```python
from build123d import *

# Parameters (mm, degrees)
SKETCH1_W           = 18
SKETCH1_H           = 56
BOSS_EXTRUDE1_DEPTH = 10
SKETCH2_W           = 6
SKETCH2_H           = 56
CUT_EXTRUDE1_DEPTH  = 1.5
HOLE1_D             = 3.242
HOLE1_DEPTH         = 6
HOLE1_CSINK_D       = 4
HOLE1_CSINK_ANGLE   = 90
HOLE1_TIP           = 0.935884786
HOLE2_D             = 3.242
HOLE2_DEPTH         = 6
HOLE2_CSINK_D       = 4
HOLE2_CSINK_ANGLE   = 90
HOLE2_TIP           = 0.935884786
HOLE3_D             = 3.242
HOLE3_DEPTH         = 6
HOLE3_CSINK_D       = 4
HOLE3_CSINK_ANGLE   = 90
HOLE3_TIP           = 0.935884786
HOLE4_D             = 3.242
HOLE4_DEPTH         = 6
HOLE4_CSINK_D       = 4
HOLE4_CSINK_ANGLE   = 90
HOLE4_TIP           = 0.935884786
SKETCH15_R          = 5
SKETCH15_R_2        = 4.5
CUT_EXTRUDE2_DEPTH  = 1
CUT_EXTRUDE3_DEPTH  = 4.33
SKETCH17_R          = 3
SKETCH17_R_2        = 2.5
CUT_EXTRUDE4_DEPTH  = 1
CUT_EXTRUDE5_DEPTH  = 3


with BuildPart() as part:
    # Sketch1 → Boss-Extrude1 (new body)
    with BuildSketch(Plane.XY.offset(9)):
        Rectangle(SKETCH1_W, SKETCH1_H)
    extrude(amount=BOSS_EXTRUDE1_DEPTH)

    # Sketch2 → Cut-Extrude1 (cut)
    with BuildSketch(Plane.XY.offset(9)):
        Rectangle(SKETCH2_W, SKETCH2_H)
    extrude(amount=CUT_EXTRUDE1_DEPTH, mode=Mode.SUBTRACT)

    # Sketch3 → Revolve1 (revolve)
    with BuildSketch(Plane(origin=(0, 0, 0), x_dir=(0, 0, -1), z_dir=(1, 0, 0)), mode=Mode.PRIVATE) as revolve1_sk:
        Polygon((-14, 12.5), (-14, 16.5), (40, 16.5), (40, 20), (45, 20), (45, 12.5), align=None)
    revolve(revolve1_sk.sketch.rotate(Axis((0, 12.5, -45), (0, 0, 1)), 270), axis=Axis((0, 12.5, -45), (0, 0, 1)))

    # Sketch4 → Revolve2 (revolve)
    with BuildSketch(Plane(origin=(0, 0, 0), x_dir=(0, 0, -1), z_dir=(1, 0, 0)), mode=Mode.PRIVATE) as revolve2_sk:
        Polygon((-14, -12.5), (-14, -8.5), (40, -8.5), (40, -5), (45, -5), (45, -12.5), align=None)
    revolve(revolve2_sk.sketch.rotate(Axis((0, -12.5, -45), (0, 0, 1)), 270), axis=Axis((0, -12.5, -45), (0, 0, 1)))

    # Sketch5 → Cut-Revolve1 (revolve, cut)
    with BuildSketch(Plane(origin=(0, 0, 0), x_dir=(0, 0, -1), z_dir=(1, 0, 0)), mode=Mode.PRIVATE) as cut_revolve1_sk:
        Polygon((-19, 22.5), (-19, 25), (-18.567, 24.567), (-10.933, 24.567), (-10.5, 25), (-10.5, 22.5), align=None)
    revolve(cut_revolve1_sk.sketch.rotate(Axis((0, 22.5, 10.5), (0, 0, 1)), 270), axis=Axis((0, 22.5, 10.5), (0, 0, 1)), mode=Mode.SUBTRACT)

    # Sketch6 → Cut-Revolve2 (revolve, cut)
    with BuildSketch(Plane(origin=(0, 0, 0), x_dir=(0, 0, -1), z_dir=(1, 0, 0)), mode=Mode.PRIVATE) as cut_revolve2_sk:
        Polygon((-19, -22.5), (-19, -20), (-18.567, -20.433), (-10.933, -20.433), (-10.5, -20), (-10.5, -22.5), align=None)
    revolve(cut_revolve2_sk.sketch.rotate(Axis((0, -22.5, 10.5), (0, 0, 1)), 270), axis=Axis((0, -22.5, 10.5), (0, 0, 1)), mode=Mode.SUBTRACT)

    # Hole1
    with Locations(Plane.ZY.offset(9)):
        with Locations((14, 22.5)):
            CounterSinkHole(HOLE1_D / 2, HOLE1_CSINK_D / 2, depth=HOLE1_DEPTH, counter_sink_angle=HOLE1_CSINK_ANGLE)
            with Locations((0, 0, -(HOLE1_DEPTH + HOLE1_TIP / 2))):  # 120° drill point
                Cone(0, HOLE1_D / 2, HOLE1_TIP, mode=Mode.SUBTRACT)

    # Hole2
    with Locations(Plane.ZY.offset(9)):
        with Locations((14, -22.5)):
            CounterSinkHole(HOLE2_D / 2, HOLE2_CSINK_D / 2, depth=HOLE2_DEPTH, counter_sink_angle=HOLE2_CSINK_ANGLE)
            with Locations((0, 0, -(HOLE2_DEPTH + HOLE2_TIP / 2))):  # 120° drill point
                Cone(0, HOLE2_D / 2, HOLE2_TIP, mode=Mode.SUBTRACT)

    # Hole3
    with Locations(Plane(origin=(9, 0, 0), x_dir=(0, 0, -1), z_dir=(1, 0, 0))):
        with Locations((-14, 22.5)):
            CounterSinkHole(HOLE3_D / 2, HOLE3_CSINK_D / 2, depth=HOLE3_DEPTH, counter_sink_angle=HOLE3_CSINK_ANGLE)
            with Locations((0, 0, -(HOLE3_DEPTH + HOLE3_TIP / 2))):  # 120° drill point
                Cone(0, HOLE3_D / 2, HOLE3_TIP, mode=Mode.SUBTRACT)

    # Hole4
    with Locations(Plane(origin=(9, 0, 0), x_dir=(0, 0, -1), z_dir=(1, 0, 0))):
        with Locations((-14, -22.5)):
            CounterSinkHole(HOLE4_D / 2, HOLE4_CSINK_D / 2, depth=HOLE4_DEPTH, counter_sink_angle=HOLE4_CSINK_ANGLE)
            with Locations((0, 0, -(HOLE4_DEPTH + HOLE4_TIP / 2))):  # 120° drill point
                Cone(0, HOLE4_D / 2, HOLE4_TIP, mode=Mode.SUBTRACT)

    # Sketch15 → Cut-Extrude2 (cut)
    with BuildSketch(Plane.XY.offset(19)):
        with Locations((0, -12.5)):
            Circle(SKETCH15_R)
        with Locations((0, -12.5)):
            Circle(SKETCH15_R_2, mode=Mode.SUBTRACT)
    extrude(amount=-CUT_EXTRUDE2_DEPTH, mode=Mode.SUBTRACT)

    # Sketch16 → Cut-Extrude3 (cut)
    with BuildSketch(Plane.XY.offset(19)):
        Polygon((-2.499926666, -12.5), (-1.249963333, -14.665), (1.249963333, -14.665), (2.499926666, -12.5), (1.249963333, -10.335), (-1.249963333, -10.335), align=None)
    extrude(amount=-CUT_EXTRUDE3_DEPTH, mode=Mode.SUBTRACT)

    # Sketch17 → Cut-Extrude4 (cut)
    with BuildSketch(Plane(origin=(9, 0, 0), x_dir=(0, 0, -1), z_dir=(1, 0, 0))):
        with Locations((-14, 12.5)):
            Circle(SKETCH17_R)
        with Locations((-14, 12.5)):
            Circle(SKETCH17_R_2, mode=Mode.SUBTRACT)
    extrude(amount=-CUT_EXTRUDE4_DEPTH, mode=Mode.SUBTRACT)

    # Sketch18 → Cut-Extrude5 (cut)
    with BuildSketch(Plane(origin=(9, 0, 0), x_dir=(0, 0, -1), z_dir=(1, 0, 0))):
        Polygon((-15.732050808, 12.5), (-14.866025404, 11), (-13.133974596, 11), (-12.267949192, 12.5), (-13.133974596, 14), (-14.866025404, 14), align=None)
    extrude(amount=-CUT_EXTRUDE5_DEPTH, mode=Mode.SUBTRACT)


solid = part.part
```
Model file for the job. Use its own axes, mm. A direction names the side the tool comes from. Round coordinates to 2 decimals unless told otherwise and drop trailing zeros. Write each loop counter-clockwise with the first axis right and the second up, starting at its lowest first coordinate (ties: lowest second). Pieces come first, ordered by that corner, then holes. Notation, with made-up numbers: (40.5, 67) -> (52.5, 67) arc R28 cw to (52.5, 90) -> close; hole circle Ø11 at (71, 26). An arc over 180 degrees is marked (long way). Answer as CSV lines item,"result".
1. Drill centre lines: line 1 (Y direction, x = 4.25, z = 14); line 2 (Z direction, x = -6.95, y = 22.5); line 3 (Y direction, x = 0, z = 14). Where is each one in solid material? Low to high.
Resolved:
line 1,"-28 to -24.12, -20.88 to 20.88, 24.12 to 28"
line 2,"9 to 12.38, 15.62 to 19"
line 3,"-28 to -24.57, -20.43 to 20.43, 24.57 to 28"
2. Slice it at B-B, the plane z = -26. List the corners of the cut face in (x, y), plus the area to 3 significant figures.
Resolved:
outline,"circle Ø8 at (0, -12.5); circle Ø8 at (0, 12.5)"
area,"101 mm²"
3. Tool access for faces 1 (the face through (-1.866, -11.402, 16.865)), 2 (the face through (-1, 20, 10.5)), 3 (the face through (3, -22, 10)), 4 (the face through (-1.63, 5.18, -42.54)), 5 (the face through (8.5, 12.6, 17)): list every direction of +Z, -Z, +X, -X, +Y, -Y with a clear straight run to the whole face (end or side of a thin tool).
Resolved:
face 1,"+Z"
face 2,"+Y"
face 3,"-Y"
face 4,"-Z"
face 5,"+X"
4. Slice it at A-A, the plane x = -6.75. List the corners of the cut face in (y, z), plus the area to 3 significant figures.
Resolved:
outline,"(-28, 9) -> (28, 9) -> (28, 19) -> (-28, 19) -> close; (-15.77, -45) -> (-9.23, -45) -> (-9.23, -40) -> (-15.77, -40) -> close; (9.23, -45) -> (15.77, -45) -> (15.77, -40) -> (9.23, -40) -> close; hole circle Ø3.24 at (-22.5, 14); hole circle Ø3.24 at (22.5, 14)"
area,"609 mm²"
5. Slice it at C-C, the plane x = 0. State how many separate pieces and enclosed holes the cut face has, plus the area to 3 significant figures.
Resolved:
separate pieces,"3"
enclosed holes,"0"
area,"1,340 mm²"
6. Mould opens along Z. For faces 6 (the face through (3, 21, 10)), 7 (the face through (-0.59, -8.04, 18.51)) say: +Z half, -Z half, draft (parallel to the pull), parting line (faces both ways), or undercut.
Resolved:
face 6,"undercut"
face 7,"draft"
7. Pin check, flat tips, straight feed: pin 1 Ø6 at (x, z) = (2, -5.5) entering from +Y; pin 2 Ø1.9 at (y, z) = (-22.5, 14) entering from +X; pin 3 Ø3.5 at (y, z) = (22.5, 14) entering from +X; pin 4 Ø5 at (y, z) = (-22.5, 14) entering from -X. Stop position of each tip, or through.
Resolved:
pin 1,"y = 16.5"
pin 2,"x = 2.61"
pin 3,"x = 8.75"
pin 4,"x = -9"
